Source: CAD feature listing. Evaluate the final solid. Frame: model axes, mm. Face numbers are marked on the shaded views. A direction names the side the tool comes from. Round coordinates to 2 decimals unless told otherwise and drop trailing zeros. Loops run counter-clockwise (first coordinate to the right, second up) from the corner with the lowest first, then second, coordinate; pieces in that order, holes last. Notation, with made-up numbers: M -3.75,-9 L 37.25,-9 A36 ccw 37.25,25 Z; hole C -7,-39 d2. An arc over 180 degrees is marked long. Answer as a JSON object with one key per item and string values.
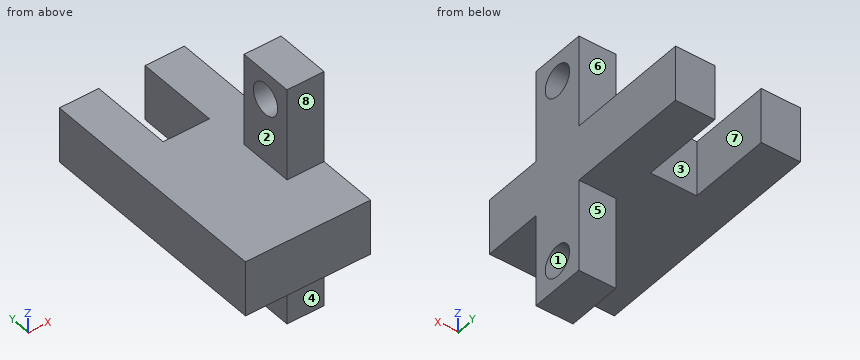
from build123d import *

# Parameters (mm, degrees)
BOSS_EXTRUDE1_DEPTH = 3
SKETCH2_W           = 26
SKETCH2_H           = 6
SKETCH2_R           = 1.7
BOSS_EXTRUDE2_DEPTH = 4


with BuildPart() as part:
    # Sketch1 → Boss-Extrude1 (new, symmetric)
    with BuildSketch(Plane.XY):
        Polygon((9.25, 0), (13.5, 0), (13.5, -26), (0, -26), (0, 0), (4.25, 0), (4.25, -9), (9.25, -9), align=None)
    extrude(amount=BOSS_EXTRUDE1_DEPTH, both=True)

    # Sketch2 → Boss-Extrude2 (add)
    with BuildSketch(Plane(origin=(13.5, 0, 0), x_dir=(0, 0, -1), z_dir=(1, 0, 0))):
        with Locations((0, -16.5)):
            Rectangle(SKETCH2_W, SKETCH2_H)
        with Locations(Location((-10, -16.5, 0), (0, 0, 90))):
            Circle(SKETCH2_R, mode=Mode.SUBTRACT)
        with Locations(Location((10, -16.5, 0), (0, 0, 90))):
            Circle(SKETCH2_R, mode=Mode.SUBTRACT)
    extrude(amount=-BOSS_EXTRUDE2_DEPTH)


solid = part.part
Item 1: Pull-direction query (Y, two-part tool) for the marked faces 1, 2 and 3; classes: pulls with the +Y half, pulls with the -Y half, needs draft (parallel to the pull), parting line crosses it, or undercut.
Answer sheet:
{"face 1": "undercut", "face 2": "needs draft", "face 3": "pulls with the +Y half"}
Item 2: Section D-D on z = -3.5. Return the cut outline in (x, y), then the cut area to 3 significant figures.
Answer sheet:
{"outline": "M 9.5,-19.5 L 13.5,-19.5 L 13.5,-13.5 L 9.5,-13.5 Z", "area": "24.0 mm²"}
Item 3: Access query for the marked faces 4, 5, 6, 7 and 8. Directions: +Z, -Z, +X, -X, +Y, -Y. A direction counts if a zero-diameter tool reaches every point of the face in a straight line with its end or side. Return the directions, or none.
Answer sheet:
{"face 4": "-Z, +X, -X, -Y", "face 5": "-Z, +X, -X, +Y", "face 6": "+Z, +X, -X, +Y", "face 7": "+Z, -Z, +Y", "face 8": "+Z, +X, -X, -Y"}
Item 4: Line query: probe 1 along Z at (x, y) = (11.4, -16.5); probe 2 along X at (y, z) = (-5, 1.75); probe 3 along X at (y, z) = (-14.25, -4.5). Output: solid intervals per line, ascending. Write a range as from..to.
Answer sheet:
{"probe 1": "z = -13..-11.7, -8.3..8.3, 11.7..13", "probe 2": "x = 0..4.25, 9.25..13.5", "probe 3": "x = 9.5..13.5"}
Item 5: Section C-C on y = -7.75. Return the cut outline in (x, z), then the cut area to 3 significant figures.
Answer sheet:
{"outline": "M 0,-3 L 4.25,-3 L 4.25,3 L 0,3 Z; M 9.25,-3 L 13.5,-3 L 13.5,3 L 9.25,3 Z", "area": "51.0 mm²"}
Item 6: Contact query for flat-ended pins moving along their axis: pin 1 Ø3 at (x, y) = (6, -19) entering from -Z; pin 2 Ø2 at (x, z) = (12.5, -9) entering from -Y; pin 3 Ø4.5 at (y, z) = (-16.5, 10) entering from -X. Output: stop coordinate, or through.
Answer sheet:
{"pin 1": "stops at z = -3", "pin 2": "stops at y = -19.5", "pin 3": "stops at x = 9.5"}
Item 7: Section B-B on y = -16.5. Return the cut outline in (x, z).
Answer sheet:
{"outline": "M 0,-3 L 9.5,-3 L 9.5,-8.3 L 13.5,-8.3 L 13.5,8.3 L 9.5,8.3 L 9.5,3 L 0,3 Z; M 9.5,-13 L 13.5,-13 L 13.5,-11.7 L 9.5,-11.7 Z; M 9.5,11.7 L 13.5,11.7 L 13.5,13 L 9.5,13 Z"}
Item 8: Section A-A on z = -10. Return the cut outline in (x, y), then the cut area to 3 significant figures.
Answer sheet:
{"outline": "M 9.5,-19.5 L 13.5,-19.5 L 13.5,-18.2 L 9.5,-18.2 Z; M 9.5,-14.8 L 13.5,-14.8 L 13.5,-13.5 L 9.5,-13.5 Z", "area": "10.4 mm²"}
